CAD build for the part. Positions are in the model's coordinates, mm. A direction names the side the tool comes from. Coordinates: 2 decimals unless noted, no trailing zeros. Order: outer loops, then holes, each group sorted by start corner. A loop starts at its lowest first (then second) coordinate and runs counter-clockwise, first axis right, second up. Notation, with made-up numbers: (78, 46) - (127, 46) arc R20 cw to (127, 82) - close; hole circle Ø2 at (76.25, 86.25). An arc over 180 degrees is marked (long way). Return JSON: item names as keys, results as strings.
from build123d import *

# Parameters (mm, degrees)
SKETCH1_W               = 40
SKETCH1_H               = 50
BOSS_EXTRUDE1_DEPTH     = 12
CUT_EXTRUDE1_DEPTH      = 35.190641995
CUT_EXTRUDE1_DEPTH_BACK = 35.190641995
SKETCH2_R               = 14
MOVE_FACE2_BY           = 60
SKETCH3_W               = 12
SKETCH3_H               = 50
BOSS_EXTRUDE2_DEPTH     = 90
CUT_EXTRUDE2_DEPTH      = 129.33160172
CUT_EXTRUDE2_DEPTH_BACK = 129.33160172
SKETCH4_R               = 14


with BuildPart() as part:
    # Sketch1 → Boss-Extrude1 (new body)
    with BuildSketch(Plane(origin=(0, 0, 0), x_dir=(1, 0, 0), z_dir=(0, 1, 0))):
        Rectangle(SKETCH1_W, SKETCH1_H)
    extrude(amount=BOSS_EXTRUDE1_DEPTH)

    # Sketch2 → Cut-Extrude1 (cut, two sides: drawn at the far end of the back side and taken through both)
    with BuildSketch(Plane(origin=(0, 12, 0), x_dir=(1, 0, 0), z_dir=(0, 1, 0)).offset(-CUT_EXTRUDE1_DEPTH_BACK)):
        with Locations(Location((0, 5, 0), (0, 0, 270))):
            Circle(SKETCH2_R)
    extrude(amount=CUT_EXTRUDE1_DEPTH + CUT_EXTRUDE1_DEPTH_BACK, mode=Mode.SUBTRACT)

    # Move Face2: a face moved outward by 60.0
    extrude(part.faces().sort_by_distance((-20, 6, 0))[0], amount=MOVE_FACE2_BY, dir=(-1, 0, 0))

    # Sketch3 → Boss-Extrude2 (add)
    with BuildSketch(Plane(origin=(0, 0, 0), x_dir=(1, 0, 0), z_dir=(0, 1, 0))):
        with Locations((-74, 0)):
            Rectangle(SKETCH3_W, SKETCH3_H)
    extrude(amount=-BOSS_EXTRUDE2_DEPTH)

    # Sketch4 → Cut-Extrude2 (cut, two sides: drawn at the far end of the back side and taken through both)
    with BuildSketch(Plane(origin=(-68, 0, 0), x_dir=(0, 0, -1), z_dir=(1, 0, 0)).offset(-CUT_EXTRUDE2_DEPTH_BACK)):
        with Locations((0, -53.54)):
            Circle(SKETCH4_R)
    extrude(amount=CUT_EXTRUDE2_DEPTH + CUT_EXTRUDE2_DEPTH_BACK, mode=Mode.SUBTRACT)


solid = part.part
Item 1: Drop flat-ended pins along their axis: P1, Ø17, axis at y = -53.54, z = 0, coming from the -X side; P2, Ø15, axis at x = -16.5, z = -5, coming from the -Y side; P3, Ø15, axis at y = -59, z = -8.5, coming from the +X side. Give the stop position or say it passes through.
Findings below:
{"P1": "passes through", "P2": "stops at y = 0", "P3": "stops at x = -68"}
Item 2: Band-saw the part on C-C, the plane z = 0. List the corners of the cut face in (x, y).
Findings below:
{"outline": "(-80, -90) - (-68, -90) - (-68, -67.54) - (-80, -67.54) - close; (-80, -39.54) - (-68, -39.54) - (-68, 0) - (-13.08, 0) - (-13.08, 12) - (-80, 12) - close; (13.08, 0) - (20, 0) - (20, 12) - (13.08, 12) - close"}
Item 3: Band-saw the part on D-D, the plane y = -83. List the corners of the cut face in (x, z), then the cut area to 3 significant figures.
Findings below:
{"outline": "(-80, -25) - (-68, -25) - (-68, 25) - (-80, 25) - close", "area": "600 mm²"}
Item 4: Wall check: L1, parallel to Z at x = -77.25, y = -53.54; L2, parallel to X at y = 4.75, z = -5; L3, parallel to Z at x = 0, y = 8.75. Give the ranges that are in metal, low to high. Write a range as [from, to].
Findings below:
{"L1": "z = [-25, -14], [14, 25]", "L2": "x = [-80, -14], [14, 20]", "L3": "z = [-25, -19], [9, 25]"}
Item 5: Which spindle directions (+Z, -Z, +X, -X, +Y, -Y) get a long thin tool onto all of the face, cutting with end or side? Do faces 4 (the flat face through (20, 6, 0)), 5 (the flat face through (-23, 0, 0)). Say none if no direction does.
Findings below:
{"face 4": "+Z, -Z, +X, +Y, -Y", "face 5": "+Z, -Z, +X, -Y"}
Item 6: Band-saw the part on A-A, the plane x = 0. List the corners of the cut face in (y, z).
Findings below:
{"outline": "(0, -25) - (12, -25) - (12, -19) - (0, -19) - close; (0, 9) - (12, 9) - (12, 25) - (0, 25) - close"}
Item 7: Mould opens along Y. For faces 1 (the flat face through (-71, -16, 25)), 2 (the cylindrical face through (-74.08, -67.21, 3.03)), 3 (the flat face through (-29, 12, 0)) say: released by +Y, released by -Y, zero draft, split by the parting line, or undercut.
Findings below:
{"face 1": "zero draft", "face 2": "undercut", "face 3": "released by +Y"}
Item 8: Band-saw the part on B-B, the plane y = -53.54. List the corners of the cut face in (x, z), then the cut area to 3 significant figures.
Findings below:
{"outline": "(-80, -25) - (-68, -25) - (-68, -14) - (-80, -14) - close; (-80, 14) - (-68, 14) - (-68, 25) - (-80, 25) - close", "area": "264 mm²"}
